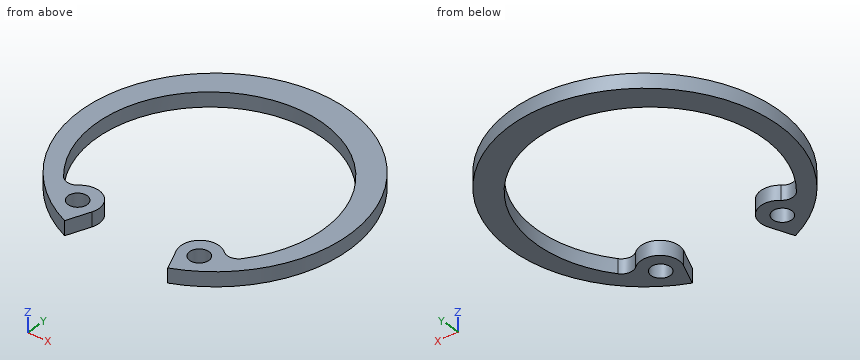
```python
from build123d import *

# Parameters (mm, degrees)
SKETCH_1_R        = 1
EXTRUDE_967_DEPTH = 1.5


with BuildPart() as part:
    # 草图1 → Extrude 967 (new body)
    with BuildSketch(Plane.XY):
        with BuildLine():
            Line((-4.368765084, -10.547131916), (-5.338433881, -12.888119479))
            ThreePointArc((-5.338433881, -12.888119479), (0, 13.95), (5.338433881, -12.888119479))
            Line((5.338433881, -12.888119479), (4.368765084, -10.547131916))
            ThreePointArc((4.368765084, -10.547131916), (5.045920823, -8.160133818), (7.524722821, -8.268947735))
            ThreePointArc((7.524722821, -8.268947735), (8.418733826, -8.556288298), (9.245939718, -8.111821553))
            ThreePointArc((9.245939718, -8.111821553), (0, 11.15), (-9.245939718, -8.111821553))
            ThreePointArc((-9.245939718, -8.111821553), (-8.418733826, -8.556288298), (-7.524722821, -8.268947735))
            ThreePointArc((-7.524722821, -8.268947735), (-5.045920823, -8.160133818), (-4.368765084, -10.547131916))
        make_face()
        with Locations((-6.298089329, -9.978680815)):
            Circle(SKETCH_1_R, mode=Mode.SUBTRACT)
        with Locations(Location((6.298089329, -9.978680815, 0), (0, 0, 180))):
            Circle(SKETCH_1_R, mode=Mode.SUBTRACT)
    extrude(amount=EXTRUDE_967_DEPTH)


solid = part.part
```
Check sheet for the modelled part. Datum: model origin and axes. Units: mm. Round coordinates to 2 decimals unless told otherwise and drop trailing zeros. Write each loop counter-clockwise with the first axis right and the second up, starting at its lowest first coordinate (ties: lowest second). Pieces come first, ordered by that corner, then holes. Notation, with made-up numbers: M 69.25,5 L 113.25,5 A14 cw 113.25,31 Z; hole C 80.5,85.5 d3. An arc over 180 degrees is marked long. Write item = value, one per line. Start each with the question number.
1. Section check B-B, the plane y = -3.25. Record the cut outline in (x, z), then the cut area to 3 significant figures.
2. Section check D-D, the plane x = 0. Record the cut outline in (y, z), then the cut area to 3 significant figures.
3. Scan lines: line 1 (X direction, y = -10.5, z = 0.65); line 2 (Y direction, x = -0.25, z = 0.7); line 3 (Y direction, x = 6, z = 0.75). Record each from-to range of solid material in increasing order. Write a range as [from, to].
4. Section check C-C, the plane z = 1. Record the cut outline in (x, y), then the cut area to 3 significant figures.
5. Section check A-A, the plane x = -9.75. Record the cut outline in (y, z), then the cut area to 3 significant figures.
Results found:
q1.outline = M -13.57,0 L -11.57,0 L -11.57,1.5 L -13.57,1.5 Z; M 11.57,0 L 13.57,0 L 13.57,1.5 L 11.57,1.5 Z
q1.area = 5.98 mm^2
q2.outline = M 11.15,0 L 13.95,0 L 13.95,1.5 L 11.15,1.5 Z
q2.area = 4.20 mm^2
q3.line_1 = [-9.18, -7.15], [-5.44, -4.35], [4.35, 5.44], [7.15, 9.18]
q3.line_2 = [11.15, 13.95]
q3.line_3 = [-12.59, -10.93], [-9.02, -7.79], [9.52, 12.59]
q4.outline = M -9.25,-8.11 A11.85 cw long 9.25,-8.11 A1.2 cw 7.52,-8.27 A2 ccw 4.37,-10.55 L 5.34,-12.89 A13.95 ccw long -5.34,-12.89 L -4.37,-10.55 A2 ccw -7.52,-8.27 A1.2 cw Z; hole C -6.3,-9.98 d2; hole C 6.3,-9.98 d2
q4.area = 169 mm^2
q5.outline = M -9.98,0 L -7.43,0 L -7.43,1.5 L -9.98,1.5 Z; M 6.03,0 L 9.98,0 L 9.98,1.5 L 6.03,1.5 Z
q5.area = 9.73 mm^2
